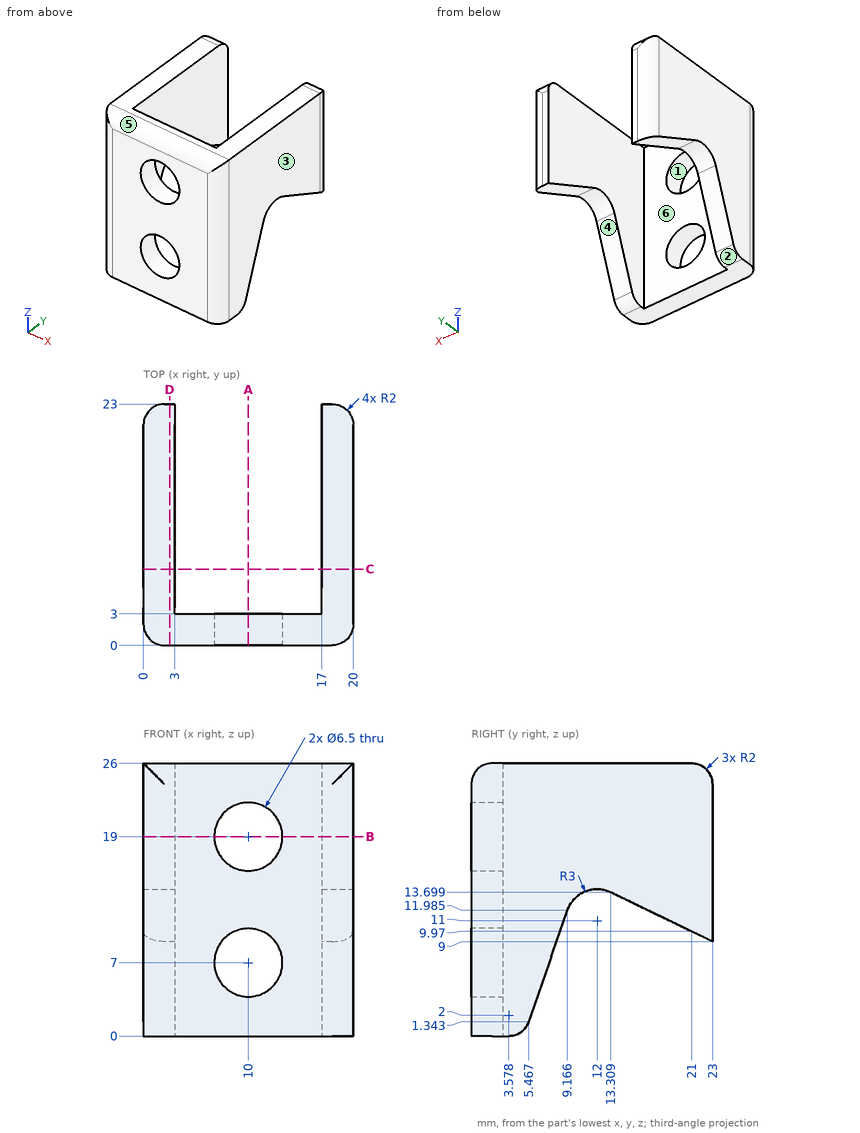
For this review, use the dimensioned drawing (mm, ordinates from the lowest corner) and the shaded views. A direction names the side the tool comes from. Give positions to 0.01 mm unless a question says otherwise; leave off trailing zeros. Order: outer loops, then holes, each group sorted by start corner. A loop starts at its lowest first (then second) coordinate and runs counter-clockwise, first axis right, second up. Notation, with made-up numbers: (73.5, 65) - (108.5, 65) arc R26 cw to (108.5, 99) - close; hole circle Ø6 at (73.25, -7.5). An arc over 180 degrees is marked (long way). Use a Markdown table: item, result. Add a question column.
(1) Mouldability with a two-part tool opening along X and no side actions: class the marked faces 1, 2 and 3 as +X half, -X half, draft (parallel to the pull), parting line (faces both ways), or undercut.
(2) Wall thickness on probe 1 along X at (y, z) = (2.4, 7); probe 2 along X at (y, z) = (8, 13.5); probe 3 along Y at (x, z) = (9.5, 10.75): over which ranges is each line inside the solid? List them lowest first. Write a range as [from, to].
(3) Machinability: for the marked faces 4, 5 and 6, which of the approach directions +Z, -Z, +X, -X, +Y, -Y give a long, thin tool a straight path to every point of the face, cutting with its end or side? Answer none if there is none.
(4) Add section B-B on z = 19. Give the boundary of the cut face in (x, y), then the cut area to 3 significant figures.
(5) Add section A-A on x = 10. Give the boundary of the cut face in (y, z).
(6) Clearance check with flat-ended pins moving along their axes: P1, Ø1, axis at x = 4.5, z = 3.5, coming from the +Y side; P2, Ø11, axis at x = 8, z = 11.5, coming from the +Y side. State where each tip first meets the part, or that it passes through.
(7) Add section D-D on x = 2.5. Give the boundary of the cut face in (y, z) (1 decimal), then the cut area to 3 significant figures.
(8) Add section C-C on y = 7.25. Give the boundary of the cut face in (x, z), then the cut area to 3 significant figures.
Report:
| question | item | result |
|---|---|---|
| 1 | face 1 | undercut |
| 1 | face 2 | draft |
| 1 | face 3 | +X half |
| 2 | probe 1 | x = [0, 6.75], [13.25, 20] |
| 2 | probe 2 | x = [0, 3], [17, 20] |
| 2 | probe 3 | y = [0, 3] |
| 3 | face 4 | -Z, +X, -X |
| 3 | face 5 | +Z, +X, -X, -Y |
| 3 | face 6 | +Z, -Z, +Y |
| 4 | outline | (0, 2) arc R2 ccw to (2, 0) - (6.75, 0) - (6.75, 3) - (3, 3) - (3, 23) - (2, 23) arc R2 ccw to (0, 21) - close; (13.25, 0) - (18, 0) arc R2 ccw to (20, 2) - (20, 21) arc R2 ccw to (18, 23) - (17, 23) - (17, 3) - (13.25, 3) - close |
| 4 | area | 157 mm² |
| 5 | outline | (0, 0) - (3, 0) - (3, 3.75) - (0, 3.75) - close; (0, 10.25) - (3, 10.25) - (3, 15.75) - (0, 15.75) - close; (0, 22.25) - (3, 22.25) - (3, 26) - (2, 26) arc R2 ccw to (0, 24) - close |
| 6 | P1 | stops at y = 3 |
| 6 | P2 | stops at y = 23 |
| 7 | outline | (0, 0) - (3.6, 0) arc R2 ccw to (5.5, 1.3) - (9.2, 12) arc R3 cw to (13.3, 13.7) - (23, 9) - (23, 24) arc R2 ccw to (21, 26) - (2, 26) arc R2 ccw to (0, 24) - close |
| 7 | area | 405 mm² |
| 8 | outline | (0, 6.47) - (3, 6.47) - (3, 26) - (0, 26) - close; (17, 6.47) - (20, 6.47) - (20, 26) - (17, 26) - close |
| 8 | area | 117 mm² |
